```python
from build123d import *

# Parameters (mm, degrees)
BASE_BLOCK_PROFILE_W        = 100
BASE_BLOCK_PROFILE_H        = 25
BASE_BLOCK_DEPTH            = 30
END_ARCH_CUT_DEPTH          = 106.148704224
END_ARCH_CUT_DEPTH_BACK     = 106.148704224
CENTER_ARCH_CUT_DEPTH       = 80.096460098
UPPER_BLOCK_PROFILE_W       = 40
UPPER_BLOCK_PROFILE_H       = 30
UPPER_BLOCK_DEPTH           = 35
SIDE_SLOT_PROFILE_W         = 5
SIDE_SLOT_PROFILE_H         = 26
SIDE_SLOT_DEPTH             = 30
TOP_BORE_PROFILE_R          = 10
TOP_BORE_20_DEPTH           = 81.156097878
BASE_NOTCH_PROFILE_W        = 20
BASE_NOTCH_PROFILE_H        = 8
BASE_NOTCH_DEPTH            = 15
TRIANGULAR_RELIEF_CUT_DEPTH = 10


with BuildPart() as part:
    # Base Block Profile → Base Block (new, symmetric)
    with BuildSketch(Plane(origin=(0, 0, 0), x_dir=(0, 0, -1), z_dir=(1, 0, 0))):
        Rectangle(BASE_BLOCK_PROFILE_W, BASE_BLOCK_PROFILE_H)
    extrude(amount=BASE_BLOCK_DEPTH, both=True)

    # End Arch Profile → End Arch Cut (cut, two sides: drawn at the far end of the back side and taken through both)
    with BuildSketch(Plane.XY.offset(50).offset(-END_ARCH_CUT_DEPTH_BACK)):
        with BuildLine():
            ThreePointArc((15, -12.5), (0, 2.5), (-15, -12.5))
            Line((-15, -12.5), (15, -12.5))
        make_face()
    extrude(amount=END_ARCH_CUT_DEPTH + END_ARCH_CUT_DEPTH_BACK, mode=Mode.SUBTRACT)

    # Center Arch Profile → Center Arch Cut (cut, through all)
    with BuildSketch(Plane(origin=(30, 0, 0), x_dir=(0, 0, -1), z_dir=(1, 0, 0))):
        with BuildLine():
            ThreePointArc((20, -12.5), (0, 7.5), (-20, -12.5))
            Line((-20, -12.5), (20, -12.5))
        make_face()
    extrude(amount=-CENTER_ARCH_CUT_DEPTH, mode=Mode.SUBTRACT)

    # Upper Block Profile → Upper Block (add, symmetric)
    with BuildSketch(Plane.XY):
        with Locations((0, 27.5)):
            Rectangle(UPPER_BLOCK_PROFILE_W, UPPER_BLOCK_PROFILE_H)
    extrude(amount=UPPER_BLOCK_DEPTH, both=True)

    # Side Slot Profile → Side Slot (cut)
    with BuildSketch(Plane(origin=(0, 42.5, 0), x_dir=(1, 0, 0), z_dir=(0, 1, 0))):
        with Locations((17.5, 0)):
            Rectangle(SIDE_SLOT_PROFILE_W, SIDE_SLOT_PROFILE_H)
    side_slot = extrude(amount=-SIDE_SLOT_DEPTH, mode=Mode.SUBTRACT)

    # Side Slot Mirror: Side Slot across plane
    add(side_slot.mirror(Plane(origin=(0, 0, 0), x_dir=(0, 0, 1), z_dir=(1, 0, 0))), mode=Mode.SUBTRACT)

    # Top Bore Profile → Top Bore Ø20 (cut, through all)
    with BuildSketch(Plane(origin=(0, 42.5, 0), x_dir=(1, 0, 0), z_dir=(0, 1, 0))):
        with Locations(Location((0, 0, 0), (0, 0, 270))):
            Circle(TOP_BORE_PROFILE_R)
    extrude(amount=-TOP_BORE_20_DEPTH, mode=Mode.SUBTRACT)

    # Base Notch Profile → Base Notch (cut)
    with BuildSketch(Plane.XY.offset(50)):
        with Locations((0, 8.5)):
            Rectangle(BASE_NOTCH_PROFILE_W, BASE_NOTCH_PROFILE_H)
    base_notch = extrude(amount=-BASE_NOTCH_DEPTH, mode=Mode.SUBTRACT)

    # Triangular Relief Profile → Triangular Relief Cut (cut, symmetric)
    with BuildSketch(Plane(origin=(0, 0, 0), x_dir=(0, 0, -1), z_dir=(1, 0, 0))):
        Polygon((-35, 12.5), (-20, 42.5), (-35, 42.5), align=None)
    triangular_relief_cut = extrude(amount=TRIANGULAR_RELIEF_CUT_DEPTH, both=True, mode=Mode.SUBTRACT)

    # Notch and Relief Mirror: Base Notch, Triangular Relief Cut across plane
    add(base_notch.mirror(Plane.XY), mode=Mode.SUBTRACT)
    add(triangular_relief_cut.mirror(Plane.XY), mode=Mode.SUBTRACT)


solid = part.part
```
Design review of the part built by this model. Coordinates are the model's own, in mm. A direction names the side the tool comes from. Coordinates: 2 decimals unless noted, no trailing zeros. Order: outer loops, then holes, each group sorted by start corner. A loop starts at its lowest first (then second) coordinate and runs counter-clockwise, first axis right, second up.
1) Mouldability with a two-part tool opening along Z and no side actions: class faces 1 (the flat face through (-17, 28, -13)), 2 (the flat face through (0, 3, 50)), 3 (the flat face through (10, 31, 29)) as +Z half, -Z half, draft (parallel to the pull), parting line (faces both ways), or undercut.
2) Take a section at D-D, the plane z = -22. Give the boundary of the cut face in (x, y).
3) Wall thickness on line 1 along X through (y, z) = (27.5, 0); line 2 along Z through (x, y) = (-19, 35.5); line 3 along Z through (x, y) = (0, 22.5): over which ranges is each line inside the solid? List them lowest first.
4) Take a section at C-C, the plane z = 0. Give the boundary of the cut face in (x, y).
5) Take a section at B-B, the plane x = 0. Give the boundary of the cut face in (y, z).
6) Take a section at A-A, the plane y = 16.5. Give the boundary of the cut face in (x, z), and give its area (3 significant figures).
7) For faces 4 (the flat face through (-10, 31, 29)), 5 (the flat face through (-17, 28, 13)), 6 (the flat face through (20, 27, 24)), list the 3-axis set-ups (+Z, -Z, +X, -X, +Y, -Y) from which the entire face can be reached by the end or side of a thin tool; tool diameter is ignored.
8) Clearance check with flat-ended pins moving along their axes: pin 1 (11 mm diameter, centred on y = 23.5, z = 23.5, fed in from +X); pin 2 (5.5 mm diameter, centred on x = 17, y = 29, fed in from +Z); pin 3 (5 mm diameter, centred on x = 8, z = 37, fed in from +Y). State where each tip first meets the part, or that it passes through.
Returned:
1. face 1: undercut
1. face 2: +Z half
1. face 3: draft
2. outline: (-30, -12.5) - (-15, -12.5) arc R15 cw to (15, -12.5) - (30, -12.5) - (30, 12.5) - (20, 12.5) - (20, 42.5) - (10, 42.5) - (10, 38.5) - (-10, 38.5) - (-10, 42.5) - (-20, 42.5) - (-20, 12.5) - (-30, 12.5) - close
3. line 1: x = -15 to -10, 10 to 15
3. line 2: z = -35 to -13, 13 to 35
3. line 3: z = -30 to -10, 10 to 30
4. outline: (-30, 7.5) - (-10, 7.5) - (-10, 42.5) - (-15, 42.5) - (-15, 12.5) - (-30, 12.5) - close; (10, 7.5) - (30, 7.5) - (30, 12.5) - (15, 12.5) - (15, 42.5) - (10, 42.5) - close
5. outline: (2.5, -50) - (4.5, -50) - (4.5, -35) - (12.5, -35) - (42.5, -20) - (42.5, -10) - (4.82, -10) arc R20 cw to (2.5, -13.23) - close; (2.5, 13.23) arc R20 cw to (4.82, 10) - (42.5, 10) - (42.5, 20) - (12.5, 35) - (4.5, 35) - (4.5, 50) - (2.5, 50) - close
6. outline: (-20, -35) - (-10, -35) - (-10, -33) - (10, -33) - (10, -35) - (20, -35) - (20, -13) - (15, -13) - (15, 13) - (20, 13) - (20, 35) - (10, 35) - (10, 33) - (-10, 33) - (-10, 35) - (-20, 35) - (-20, 13) - (-15, 13) - (-15, -13) - (-20, -13) - close; hole circle Ø20 at (0, 0)
6. area: 2,150 mm2
7. face 4: +Z, +Y
7. face 5: -X, +Y
7. face 6: +Z, -Z, +X, +Y
8. pin 1: stops at x = 20
8. pin 2: stops at z = 35
8. pin 3: stops at y = 13.5
